```python
from build123d import *

# Parameters (mm, degrees)
GB_6728_1986_150_X_150_X_5_1_DEPTH = 2700


with BuildPart() as part:
    # Sketch1 → Gb／6728-1986方形空心型钢 150 X 150 X 5(1) (new body)
    with BuildSketch(Plane.YZ.offset(-1350)):
        with BuildLine():
            Line((-65, -75), (65, -75))
            ThreePointArc((65, -75), (72.071067812, -72.071067812), (75, -65))
            Line((75, -65), (75, 65))
            ThreePointArc((75, 65), (72.071067812, 72.071067812), (65, 75))
            Line((65, 75), (-65, 75))
            ThreePointArc((-65, 75), (-72.071067812, 72.071067812), (-75, 65))
            Line((-75, 65), (-75, -65))
            ThreePointArc((-75, -65), (-72.071067812, -72.071067812), (-65, -75))
        make_face()
        with BuildLine():
            Line((-65, -70), (65, -70))
            ThreePointArc((65, -70), (68.535533906, -68.535533906), (70, -65))
            Line((70, -65), (70, 65))
            ThreePointArc((70, 65), (68.535533906, 68.535533906), (65, 70))
            Line((65, 70), (-65, 70))
            ThreePointArc((-65, 70), (-68.535533906, 68.535533906), (-70, 65))
            Line((-70, 65), (-70, -65))
            ThreePointArc((-70, -65), (-68.535533906, -68.535533906), (-65, -70))
        make_face(mode=Mode.SUBTRACT)
    extrude(amount=GB_6728_1986_150_X_150_X_5_1_DEPTH)


solid = part.part
```
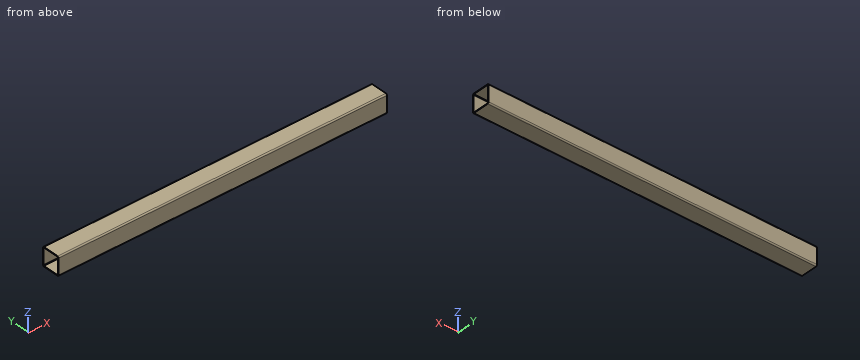
The listing builds one solid part. Answer for the finished solid, in the listing's coordinates (mm). Give positions to 0.01 mm unless a question says otherwise; leave off trailing zeros. Order: outer loops, then holes, each group sorted by start corner. A loop starts at its lowest first (then second) coordinate and runs counter-clockwise, first axis right, second up. Notation, with made-up numbers: (14, 44) -> (28, 44) arc R24 ccw to (28, 75) -> close; hole circle Ø9 at (33.25, -19). An arc over 180 degrees is marked (long way). One line per item, written item: value.
1) Find section A-A, the plane z = 17. Determine the outline of the cut face in (x, y).
Reported:
outline: (-1350, -75) -> (1350, -75) -> (1350, -70) -> (-1350, -70) -> close; (-1350, 70) -> (1350, 70) -> (1350, 75) -> (-1350, 75) -> close
2) Find section C-C, the plane x = 687.5. Determine the outline of the cut face in (y, z), plus the area to 3 significant figures.
Reported:
outline: (-75, -65) arc R10 ccw to (-65, -75) -> (65, -75) arc R10 ccw to (75, -65) -> (75, 65) arc R10 ccw to (65, 75) -> (-65, 75) arc R10 ccw to (-75, 65) -> close; hole (-70, -65) arc R5 ccw to (-65, -70) -> (65, -70) arc R5 ccw to (70, -65) -> (70, 65) arc R5 ccw to (65, 70) -> (-65, 70) arc R5 ccw to (-70, 65) -> close
area: 2,840 mm^2
3) Find the intervals of material crossed by line 1 (Z direction, x = -975.5, y = 44), in increasing order.
Reported:
line 1: z = -75 to -70, 70 to 75
